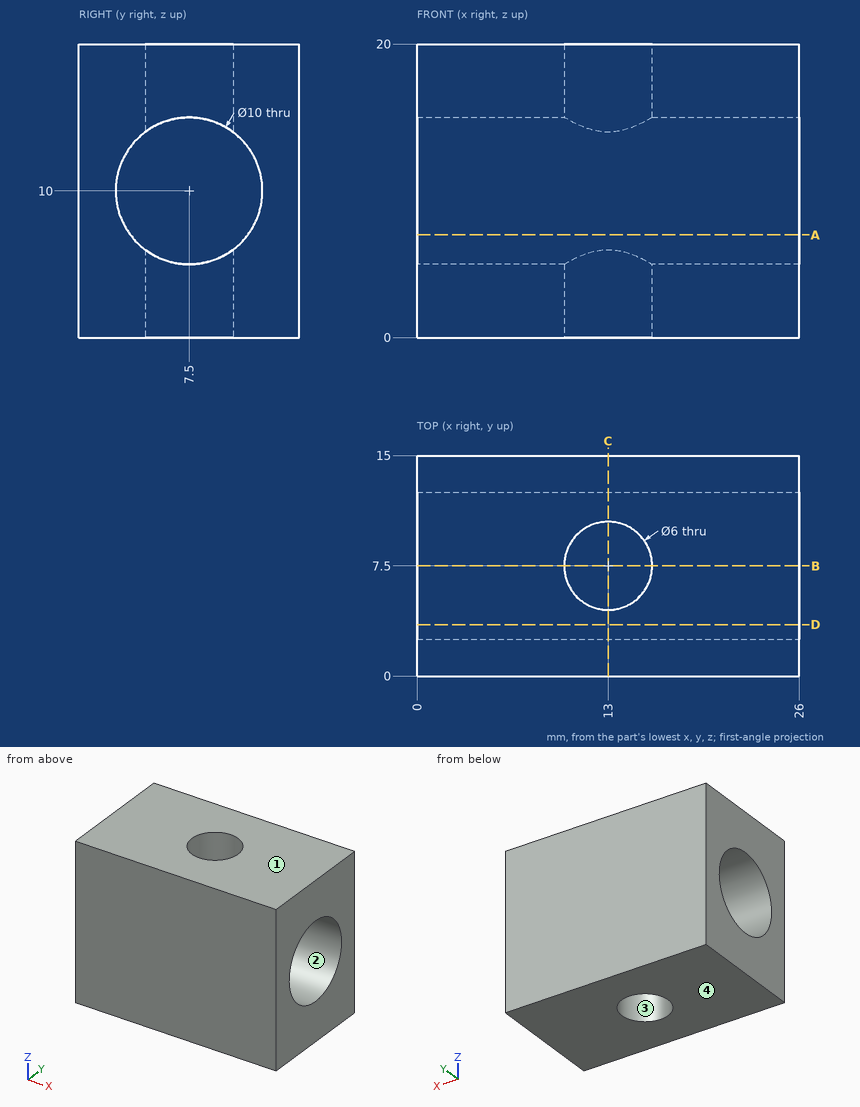
Could you check a few things on this drawing? It's one solid part, dimensions in mm from its lowest x, y, z. Round coordinates to 2 decimals unless told otherwise and drop trailing zeros. Order: outer loops, then holes, each group sorted by start corner. A loop starts at its lowest first (then second) coordinate and runs counter-clockwise, first axis right, second up.
Q1. Imagine slicing it at B-B, the plane y = 7.5. List the corners of the cut face in (x, z) for me, then the cut area to 3 significant figures.
Geometry says:
outline: (0, 0) - (10, 0) - (10, 5) - (0, 5) - close; (0, 15) - (10, 15) - (10, 20) - (0, 20) - close; (16, 0) - (26, 0) - (26, 5) - (16, 5) - close; (16, 15) - (26, 15) - (26, 20) - (16, 20) - close
area: 200 mm2
Q2. I'm going to push a flat-ended pin straight in: P1, Ø3.5, axis at x = 13, y = 7.5, coming from the -Z side. Where does the tip first touch, or does it pass through?
Geometry says:
P1: passes through
Q3. Imagine slicing it at A-A, the plane z = 7. List the corners of the cut face in (x, y) for me, then the cut area to 3 significant figures.
Geometry says:
outline: (0, 0) - (26, 0) - (26, 3.5) - (0, 3.5) - close; (0, 11.5) - (26, 11.5) - (26, 15) - (0, 15) - close
area: 182 mm2
Q4. Imagine slicing it at C-C, the plane x = 13. List the corners of the cut face in (y, z) for me.
Geometry says:
outline: (0, 0) - (4.5, 0) - (4.5, 6) arc R5 cw to (4.5, 14) - (4.5, 20) - (0, 20) - close; (10.5, 0) - (15, 0) - (15, 20) - (10.5, 20) - (10.5, 14) arc R5 cw to (10.5, 6) - close
Q5. Please list where these lines run through material, in increasing order: probe 1 along Y at (x, z) = (13, 2); probe 2 along Z at (x, y) = (3.25, 4.5); probe 3 along Z at (x, y) = (17.75, 7.5).
Geometry says:
probe 1: y = 0 to 4.5, 10.5 to 15
probe 2: z = 0 to 6, 14 to 20
probe 3: z = 0 to 5, 15 to 20
Q6. Imagine slicing it at D-D, the plane y = 3.5. List the corners of the cut face in (x, z) for me, then the cut area to 3 significant figures.
Geometry says:
outline: (0, 0) - (26, 0) - (26, 7) - (0, 7) - close; (0, 13) - (26, 13) - (26, 20) - (0, 20) - close
area: 364 mm2
Q7. Thinking about a two-plate mould opening in Z: for the marked faces 1, 2, 3 and 4, which applies, released by +Z, released by -Z, zero draft, split by the parting line, or undercut?
Geometry says:
face 1: released by +Z
face 2: undercut
face 3: zero draft
face 4: released by -Z
